Build history of the part. All positions in model axes, mm. A direction names the side the tool comes from. Coordinates: 2 decimals unless noted, no trailing zeros. Loops run counter-clockwise (first coordinate to the right, second up) from the corner with the lowest first, then second, coordinate; pieces in that order, holes last.
(1) Slice it at A-A (z = -1.5). Give the cut face in (x, y).
(2) Slice it at C-C (x = 95). Give the cut face in (y, z), and give its area (3 significant figures).
(3) Two-plate mould, pull along X, no slides. Class faces 6 (the face through (0, 19, 3)), 7 (the face through (32, 19, -2)), 8 (the face through (94.479, 32.966, 3.042)), 9 (the face through (55, 0, -36)): pulls with the +X half, pulls with the -X half, needs draft (parallel to the pull), parting line crosses it, or undercut.
(4) Slice it at D-D (y = 16). Give the cut face in (x, z), and give its area (3 significant figures).
(5) Wall check: L1, parallel to Y at x = 15, z = 2.25; L2, parallel to X at y = 2.5, z = -4.5; L3, parallel to X at y = 11, z = -36. Give the ranges that are in metal, low to high.
(6) Flat gauge pins, fed straight in: P1, Ø12, axis at y = 4.5, z = -12, coming from the -X side; P2, Ø9, axis at x = 95, y = 29, coming from the -Z side; P3, Ø2, axis at y = 33, z = -38.5, coming from the +X side; P4, Ø21, axis at y = 26, z = -10, coming from the +X side. Where does each tip first touch, or does it go through?
(7) Tool access for faces 1 (the face through (78, 19, -2)), 2 (the face through (99, 20, 0)), 3 (the face through (91, 10, 3)), 4 (the face through (11, 20, 0)), 5 (the face through (16, 20, 6)): list every direction of +Z, -Z, +X, -X, +Y, -Y with a clear straight run to the whole face (end or side of a thin tool).
(8) Slice it at B-B (y = 29). Give the cut face in (x, z).
from build123d import *

# Parameters (mm, degrees)
BASE_PLATE_SKETCH_W       = 110
BASE_PLATE_SKETCH_H       = 39
BASE_PLATE_110X39X6_DEPTH = 6
SADDLE_BODY_39_DEPTH      = 39
SADDLE_CUTOUT_SKETCH_W    = 46
SADDLE_CUTOUT_SKETCH_H    = 6
SADDLE_CUTOUT_DEPTH       = 39
FLANGE_HOLES_SKETCH_R     = 4
FLANGE_HOLES_4X_8_DEPTH   = 39


with BuildPart() as part:
    # Base Plate Sketch → Base Plate 110x39x6 (new body)
    with BuildSketch(Plane.XY):
        with Locations((55, 19.5)):
            Rectangle(BASE_PLATE_SKETCH_W, BASE_PLATE_SKETCH_H)
    extrude(amount=BASE_PLATE_110X39X6_DEPTH)

    # Saddle Body Profile → Saddle Body 39 (add)
    with BuildSketch(Plane.XZ):
        with BuildLine():
            Line((32, -10), (32, 0))
            Line((32, 0), (22.5, 0))
            Line((22.5, 0), (22.5, -26.5))
            Line((22.5, -26.5), (42, -46))
            Line((42, -46), (55, -46))
            Line((55, -46), (55, -33))
            ThreePointArc((55, -33), (38.736544033, -26.263455967), (32, -10))
        make_face()
        with BuildLine():
            Line((87.5, 0), (78, 0))
            Line((78, 0), (78, -10))
            ThreePointArc((78, -10), (71.263455967, -26.263455967), (55, -33))
            Line((55, -33), (55, -46))
            Line((55, -46), (68, -46))
            Line((68, -46), (87.5, -26.5))
            Line((87.5, -26.5), (87.5, 0))
        make_face()
    extrude(amount=-SADDLE_BODY_39_DEPTH)

    # Saddle Cutout Sketch → Saddle Cutout (cut)
    with BuildSketch(Plane.XZ):
        with Locations((55, 3)):
            Rectangle(SADDLE_CUTOUT_SKETCH_W, SADDLE_CUTOUT_SKETCH_H)
    extrude(amount=-SADDLE_CUTOUT_DEPTH, mode=Mode.SUBTRACT)

    # Flange Holes Sketch → Flange Holes 4xØ8 (cut)
    with BuildSketch(Plane.XY.offset(6)):
        with Locations((15, 29)):
            Circle(FLANGE_HOLES_SKETCH_R)
        with Locations((15, 10)):
            Circle(FLANGE_HOLES_SKETCH_R)
        with Locations((95, 29)):
            Circle(FLANGE_HOLES_SKETCH_R)
        with Locations((95, 10)):
            Circle(FLANGE_HOLES_SKETCH_R)
    extrude(amount=-FLANGE_HOLES_4X_8_DEPTH, mode=Mode.SUBTRACT)


solid = part.part
Response values:
1. outline: (22.5, 0) - (32, 0) - (32, 39) - (22.5, 39) - close; (78, 0) - (87.5, 0) - (87.5, 39) - (78, 39) - close
2. outline: (0, 0) - (6, 0) - (6, 6) - (0, 6) - close; (14, 0) - (25, 0) - (25, 6) - (14, 6) - close; (33, 0) - (39, 0) - (39, 6) - (33, 6) - close
2. area: 138 mm2
3. face 6: pulls with the -X half
3. face 7: undercut
3. face 8: undercut
3. face 9: needs draft
4. outline: (0, 0) - (22.5, 0) - (22.5, -26.5) - (42, -46) - (68, -46) - (87.5, -26.5) - (87.5, 0) - (110, 0) - (110, 6) - (78, 6) - (78, -10) arc R23 cw to (32, -10) - (32, 6) - (0, 6) - close
4. area: 1,700 mm2
5. L1: y = 0 to 6, 14 to 25, 33 to 39
5. L2: x = 22.5 to 32, 78 to 87.5
5. L3: x = 32 to 78
6. P1: stops at x = 22.5
6. P2: stops at z = 0
6. P3: stops at x = 76.5
6. P4: stops at x = 110
7. face 1: +Z, +Y, -Y
7. face 2: -Z, +X, +Y, -Y
7. face 3: +Z, -Z
7. face 4: -Z, -X, +Y, -Y
7. face 5: +Z, +X, -X, +Y, -Y
8. outline: (0, 0) - (11, 0) - (11, 6) - (0, 6) - close; (19, 0) - (22.5, 0) - (22.5, -26.5) - (42, -46) - (68, -46) - (87.5, -26.5) - (87.5, 0) - (91, 0) - (91, 6) - (78, 6) - (78, -10) arc R23 cw to (32, -10) - (32, 6) - (19, 6) - close; (99, 0) - (110, 0) - (110, 6) - (99, 6) - close
